For this review, take the finished solid that the model builds, in its own axes (mm). Face numbers are marked on the shaded views. A direction names the side the tool comes from. Round coordinates to 2 decimals unless told otherwise and drop trailing zeros. Order: outer loops, then holes, each group sorted by start corner. A loop starts at its lowest first (then second) coordinate and runs counter-clockwise, first axis right, second up. Notation, with made-up numbers: M 21,-6 L 29,-6 A24 ccw 29,20 Z; hole C 76,33.5 d2. An arc over 180 degrees is marked long. Answer in a Markdown table with one row per item. Add a question column.
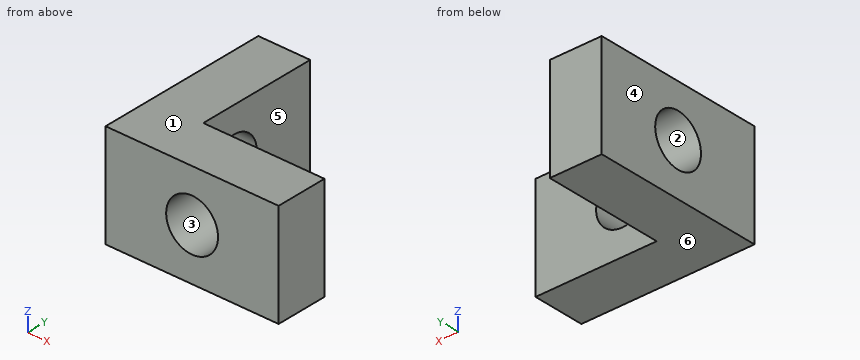
```python
from build123d import *

# Parameters (mm, degrees)
EXTRUDE_4_DEPTH     = 6
SKETCH_7_R          = 1.5
CUT_EXTRUDE_3_DEPTH = 14.601470509
SKETCH_8_R          = 1.5
CUT_EXTRUDE_4_DEPTH = 14.601470509


with BuildPart() as part:
    # 草图6 → 凸台-拉伸4 (new body)
    with BuildSketch(Plane.XY):
        Polygon((0, 0), (10, 0), (10, 3), (3, 3), (3, 10), (0, 10), align=None)
    extrude(amount=EXTRUDE_4_DEPTH)

    # 草图7 → 切除-拉伸3 (cut, through all)
    with BuildSketch(Plane(origin=(3, 0, 0), x_dir=(0, 0, -1), z_dir=(1, 0, 0))):
        with Locations(Location((-3, 5, 0), (0, 0, 90))):
            Circle(SKETCH_7_R)
    extrude(amount=-CUT_EXTRUDE_3_DEPTH, mode=Mode.SUBTRACT)

    # 草图8 → 切除-拉伸4 (cut, through all)
    with BuildSketch(Plane(origin=(0, 3, 0), x_dir=(1, 0, 0), z_dir=(0, 1, 0))):
        with Locations(Location((5, -3, 0), (0, 0, 180))):
            Circle(SKETCH_8_R)
    extrude(amount=-CUT_EXTRUDE_4_DEPTH, mode=Mode.SUBTRACT)


solid = part.part
```
1. Clearance check with flat-ended pins moving along their axes: pin 1 Ø2.5 at (x, z) = (5, 3) entering from +Y; pin 2 Ø1.8 at (x, z) = (6, 3) entering from +Y. State where each tip first meets the part, or that it passes through.
2. For the marked faces 5 and 6, list the 3-axis set-ups (+Z, -Z, +X, -X, +Y, -Y) from which the entire face can be reached by the end or side of a thin tool; tool diameter is ignored.
3. To check wall thickness, follow probe 1 along Y at (x, z) = (1.5, 2.9); probe 2 along Z at (x, y) = (5, 1.25); probe 3 along Y at (x, z) = (3.25, 0.8). State the ranges of each line that lie inside material, in increasing order. Write a range as [from, to].
4. The part is to be moulded in two halves that separate along Z. For the marked faces 1, 2, 3 and 4, say which applies: pulls with the +Z half, pulls with the -Z half, needs draft (parallel to the pull), parting line crosses it, or undercut.
5. Consider section D-D on y = 2.5. Write out the cut boundary in (x, z), plus the area to 3 significant figures.
6. Consider section A-A on z = 3. Write out the cut boundary in (x, y), plus the area to 3 significant figures.
7. Consider section B-B on x = 5. Write out the cut boundary in (y, z), plus the area to 3 significant figures.
Solved:
| question | item | result |
|---|---|---|
| 1 | pin 1 | passes through |
| 1 | pin 2 | stops at y = 3 |
| 2 | face 5 | +Z, -Z, +X, +Y |
| 2 | face 6 | -Z, +X, -X, +Y, -Y |
| 3 | probe 1 | y = [0, 3.5], [6.5, 10] |
| 3 | probe 2 | z = [0, 1.5], [4.5, 6] |
| 3 | probe 3 | y = [0, 3] |
| 4 | face 1 | pulls with the +Z half |
| 4 | face 2 | undercut |
| 4 | face 3 | undercut |
| 4 | face 4 | needs draft |
| 5 | outline | M 0,0 L 10,0 L 10,6 L 0,6 Z; hole C 5,3 d3 |
| 5 | area | 52.9 mm^2 |
| 6 | outline | M 0,0 L 3.5,0 L 3.5,3 L 3,3 L 3,3.5 L 0,3.5 Z; M 0,6.5 L 3,6.5 L 3,10 L 0,10 Z; M 6.5,0 L 10,0 L 10,3 L 6.5,3 Z |
| 6 | area | 33.0 mm^2 |
| 7 | outline | M 0,0 L 3,0 L 3,1.5 L 0,1.5 Z; M 0,4.5 L 3,4.5 L 3,6 L 0,6 Z |
| 7 | area | 9.00 mm^2 |
